Check sheet for the modelled part. Datum: model origin and axes. Units: mm. Face numbers are marked on the shaded views. Round coordinates to 2 decimals unless told otherwise and drop trailing zeros. Write each loop counter-clockwise with the first axis right and the second up, starting at its lowest first coordinate (ties: lowest second). Pieces come first, ordered by that corner, then holes. Notation, with made-up numbers: (-21, 33.25) -> (13, 33.25) arc R13 cw to (13, 48.25) -> close; hole circle Ø4 at (55.25, 87.25). An arc over 180 degrees is marked (long way). Answer as a JSON object with one key per item and string values. Group by question number.
```python
from build123d import *

# Parameters (mm, degrees)
SKETCH_1_W              = 13
SKETCH_1_H              = 13
EXTRUDE_1_DEPTH         = 6
HOLE_WIZARD_3_5_3_5_1_D = 3.5
CHAMFER_1_SIZE          = 1


with BuildPart() as part:
    # 草图1 → 凸台-拉伸1 (new body)
    with BuildSketch(Plane(origin=(0, 0, 0), x_dir=(1, 0, 0), z_dir=(0, 1, 0))):
        Rectangle(SKETCH_1_W, SKETCH_1_H)
    extrude(amount=EXTRUDE_1_DEPTH)

    # Ø3.5 (3.5) 直径孔1 (through all)
    with Locations(Plane(origin=(0, 6, 0), x_dir=(1, 0, 0), z_dir=(0, 1, 0))):
        with Locations((0, 0)):
            Hole(HOLE_WIZARD_3_5_3_5_1_D / 2)

    # 倒角1
    chamfer_1_edges = [part.edges().sort_by_distance(p)[0] for p in [
        (6.5, 3, 6.5),
        (-6.5, 3, 6.5),
        (-6.5, 3, -6.5),
        (6.5, 3, -6.5),
    ]]
    chamfer(chamfer_1_edges, length=CHAMFER_1_SIZE)


solid = part.part
```
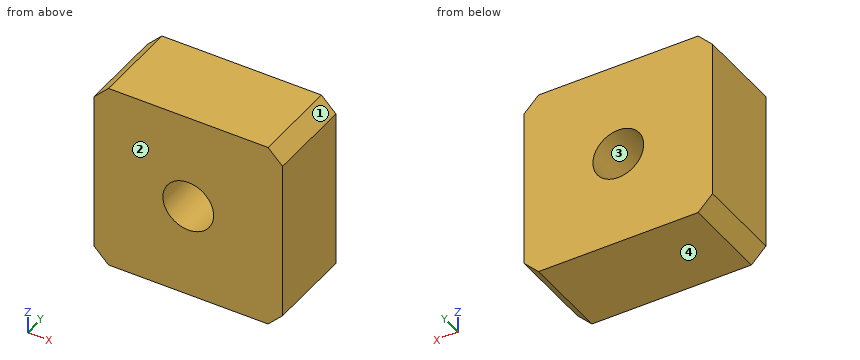
(1) Section check C-C on y = 1.3. Record the cut outline in (x, z), then the cut area to 3 significant figures.
(2) Scan lines: line 1 along Z through (x, y) = (0, 1.3); line 2 along X through (y, z) = (4.2, -1.5); line 3 along Z through (x, y) = (1, 3.1). Record each from-to range of solid material in increasing order.
(3) Section check B-B on x = 0. Record the cut outline in (y, z), then the cut area to 3 significant figures.
(4) Release check for a two-part mould opening along Z. For the marked faces 1, 2, 3 and 4 record: pulls with the +Z half, pulls with the -Z half, needs draft (parallel to the pull), parting line crosses it, or undercut.
(5) Section check A-A on z = 0. Record the cut outline in (x, y).
Data:
{
 "1": {"outline": "(-6.5, -5.5) -> (-5.5, -6.5) -> (5.5, -6.5) -> (6.5, -5.5) -> (6.5, 5.5) -> (5.5, 6.5) -> (-5.5, 6.5) -> (-6.5, 5.5) -> close; hole circle Ø3.5 at (0, 0)", "area": "157 mm²"},
 "2": {"line 1": "z = -6.5 to -1.75, 1.75 to 6.5", "line 2": "x = -6.5 to -0.9, 0.9 to 6.5", "line 3": "z = -6.5 to -1.44, 1.44 to 6.5"},
 "3": {"outline": "(0, -6.5) -> (6, -6.5) -> (6, -1.75) -> (0, -1.75) -> close; (0, 1.75) -> (6, 1.75) -> (6, 6.5) -> (0, 6.5) -> close", "area": "57.0 mm²"},
 "4": {"face 1": "pulls with the +Z half", "face 2": "needs draft", "face 3": "undercut", "face 4": "pulls with the -Z half"},
 "5": {"outline": "(-6.5, 0) -> (-1.75, 0) -> (-1.75, 6) -> (-6.5, 6) -> close; (1.75, 0) -> (6.5, 0) -> (6.5, 6) -> (1.75, 6) -> close"}
}
